```python
from build123d import *

# Parameters (mm, degrees)
SKETCH5_R           = 16
BOSS_EXTRUDE1_DEPTH = 60
SKETCH6_R           = 9
BOSS_EXTRUDE2_DEPTH = 70
BOSS_EXTRUDE3_START = 100
SKETCH7_R           = 16
BOSS_EXTRUDE3_DEPTH = 100
SKETCH8_R           = 11.952224842
BOSS_EXTRUDE4_DEPTH = 5
LPATTERN1_COUNT     = 2
LPATTERN1_PITCH     = 40


with BuildPart() as part:
    # Sketch5 → Boss-Extrude1 (new body)
    with BuildSketch(Plane.XY):
        with Locations((-19.20096517, 5.868531988)):
            Circle(SKETCH5_R)
    extrude(amount=-BOSS_EXTRUDE1_DEPTH)

    # Sketch6 → Boss-Extrude2 (add)
    with BuildSketch(Plane(origin=(0, 0, -60), x_dir=(-1, 0, 0), z_dir=(0, 0, -1))):
        with Locations((19.20096517, 5.868531988)):
            Circle(SKETCH6_R)
    extrude(amount=BOSS_EXTRUDE2_DEPTH)

    # Sketch7 → Boss-Extrude3 (add)
    with BuildSketch(Plane.XY.offset(BOSS_EXTRUDE3_START)):
        with Locations((-19.20096517, 5.868531988)):
            Circle(SKETCH7_R)
    extrude(amount=-BOSS_EXTRUDE3_DEPTH)

    # Sketch8 → Boss-Extrude4 (add)
    with BuildSketch(Plane(origin=(0, 0, -130), x_dir=(-1, 0, 0), z_dir=(0, 0, -1))):
        with Locations((19.20096517, 5.868531988)):
            Circle(SKETCH8_R)
    boss_extrude4 = extrude(amount=BOSS_EXTRUDE4_DEPTH)

    # LPattern1: Boss-Extrude4 ×2
    with Locations(*[(0, 0, i * LPATTERN1_PITCH) for i in range(1, LPATTERN1_COUNT)]):
        add(boss_extrude4)


solid = part.part
```
Work out the finished part from the listing and answer in its coordinate system (mm). A direction names the side the tool comes from. Give positions to 0.01 mm unless a question says otherwise; leave off trailing zeros. Order: outer loops, then holes, each group sorted by start corner. A loop starts at its lowest first (then second) coordinate and runs counter-clockwise, first axis right, second up. Notation, with made-up numbers: M 75.5,79.25 L 86.5,79.25 A34 ccw 86.5,117.25 Z; hole C 68,10 d5. An arc over 180 degrees is marked long. Return JSON: item names as keys, results as strings.
1) A tool of negligible diameter and unlimited length cuts with its end or side. For faces 4 (the flat face through (-21, 15, -95)), 5 (the cylindrical face through (-35.185, 6.572, 21.12)), 6 (the cylindrical face through (-7.26, 6.39, -92.46)), from which of +Z, -Z, +X, -X, +Y, -Y can it reach the whole face along a straight path? Write none if from no direction.
Resolved:
{"face 4": "none", "face 5": "+Z, -Z", "face 6": "-Z"}
2) Section B-B, the plane y = 2 is taken. Write down the section's boundary in (x, z).
Resolved:
{"outline": "M -34.73,-60 L -27.33,-60 L -27.33,-90 L -30.51,-90 L -30.51,-95 L -27.33,-95 L -27.33,-130 L -30.51,-130 L -30.51,-135 L -7.89,-135 L -7.89,-130 L -11.07,-130 L -11.07,-95 L -7.89,-95 L -7.89,-90 L -11.07,-90 L -11.07,-60 L -3.68,-60 L -3.68,100 L -34.73,100 Z"}
3) Straight lines are drawn through the part: line 1 along Z through (x, y) = (-10, 3.5); line 2 along Z through (x, y) = (-14, 17); line 3 along X through (y, z) = (6, -122). For each, find the intervals that lie inside material, in ascending order. Write a range as [from, to].
Resolved:
{"line 1": "[-135, -130], [-95, -90], [-60, 100]", "line 2": "[-60, 100]", "line 3": "[-28.2, -10.2]"}
4) Each of these flat-tipped pins is pushed along its axis until it touches: pin 1 (2 mm diameter, centred on y = 8.5, z = -100.5, fed in from -X); pin 2 (1.5 mm diameter, centred on x = -26.5, z = -97.5, fed in from -Y); pin 3 (1 mm diameter, centred on y = -3.5, z = 6.5, fed in from +X). Where does it stop, or does it pass through?
Resolved:
{"pin 1": "x = -28.05", "pin 2": "y = -0.3", "pin 3": "x = -5.88"}
5) Section C-C, the plane z = -68.5 is taken. Write down the section's boundary in (x, y), plus the area to 3 significant figures.
Resolved:
{"outline": "C -19.2,5.87 d18", "area": "254 mm^2"}
6) Section A-A, the plane x = -14 is taken. Write down the section's boundary in (y, z).
Resolved:
{"outline": "M -9.26,-60 L -1.48,-60 L -1.48,-90 L -4.89,-90 L -4.89,-95 L -1.48,-95 L -1.48,-130 L -4.89,-130 L -4.89,-135 L 16.63,-135 L 16.63,-130 L 13.21,-130 L 13.21,-95 L 16.63,-95 L 16.63,-90 L 13.21,-90 L 13.21,-60 L 21,-60 L 21,100 L -9.26,100 Z"}
7) For a pull along Z with two mould halves and no side action, classify faces 1 (the cylindrical face through (-7.26, 6.39, -132.46)), 2 (the flat face through (-21, 15, -90)), 3 (the flat face through (-19, 6, 100)) as +Z half, -Z half, draft (parallel to the pull), parting line (faces both ways), or undercut.
Resolved:
{"face 1": "draft", "face 2": "undercut", "face 3": "+Z half"}
